Source: CAD feature listing. Evaluate the final solid. Frame: model axes, mm. Face numbers are marked on the shaded views. A direction names the side the tool comes from. Give positions to 0.01 mm unless a question says otherwise; leave off trailing zeros. Order: outer loops, then holes, each group sorted by start corner. A loop starts at its lowest first (then second) coordinate and runs counter-clockwise, first axis right, second up. Notation, with made-up numbers: M -30,-24.75 L -14,-24.75 A22 ccw -14,2.25 Z; hole C 0,61 d3. An arc over 180 degrees is marked long. Use CSV: the item, a comma, the result in double quotes. Start each with the question number.
Item 1: Section query B-B on y = 67. Return loops of the section in (x, z), and give its area (3 significant figures).
Item 2: Pull-direction query (X, two-part tool) for the marked faces 4, 5, 6 and 7; classes: +X half, -X half, draft (parallel to the pull), parting line (faces both ways), or undercut.
Item 3: Access query for the marked faces 1, 2 and 3. Directions: +Z, -Z, +X, -X, +Y, -Y. A direction counts if a zero-diameter tool reaches every point of the face in a straight line with its end or side. Return the directions, or none.
Item 4: Section query D-D on x = 133.5. Return loops of the section in (y, z).
Item 5: First-contact query: pin 1 (12 mm diameter, centred on x = 128.5, y = 21, fed in from -Z); pin 2 (18.5 mm diameter, centred on y = 20, z = 11.5, fed in from +X); pin 3 (15 mm diameter, centred on x = 144, z = 32.5, fed in from +Y); pin 4 (2 mm diameter, centred on x = 63.5, z = 54, fed in from +Y). Flat tips, straight axial feed; report the tip coordinate or a pass-through.
Item 6: Ray query, probe 1 along Z at (x, y) = (62.5, 22.5); probe 2 along Z at (x, y) = (96.5, 29.5); probe 3 along Y at (x, z) = (90, 66). Return the intervals inside material, ascending. Write a range as from..to.
Item 7: Section query C-C on x = 80.5. Return loops of the section in (y, z).
Item 8: Section query A-A on z = 41. Return loops of the section in (x, y), and give its area (4 significant figures).
from build123d import *

# Parameters (mm, degrees)
BASE_BLOCK_DEPTH       = 82
POCKET_1_SKETCH_W      = 82
POCKET_1_SKETCH_H      = 15
POCKET_CUT_1_DEPTH     = 82
POCKET_2_SKETCH_W      = 12
POCKET_2_SKETCH_H      = 82
POCKET_CUT_2_DEPTH     = 82
PAD_SKETCH_W           = 12
PAD_SKETCH_H           = 15
FULL_WIDTH_PAD_DEPTH   = 82
LUG_1_DEPTH            = 22
LUG_START              = -22
LUG_2_DEPTH            = 22
WEB_1_DEPTH            = 12
WEB_2_DEPTH            = 12
WEB_3_DEPTH            = 12
WEB_4_DEPTH            = 12
LUG_BORE_SKETCH_R      = 14
LUG_BORE_DEPTH         = 100
EAR_BOSS_DEPTH         = 15
EAR_HOLE_SKETCH_R      = 11
EAR_HOLE_DEPTH         = 15
SIDE_BOSS_DEPTH        = 10
BEARING_SEAT_CUT_DEPTH = 28


with BuildPart() as part:
    # Base Profile Sketch → Base Block (new body)
    with BuildSketch(Plane.XY):
        Polygon((0, 15), (0, 0), (140, 0), (140, 30), (128, 30), (128, 15), (18, 14), (18, 54), (0, 54), align=None)
    extrude(amount=BASE_BLOCK_DEPTH)

    # Pocket 1 Sketch → Pocket Cut 1 (cut)
    with BuildSketch(Plane.ZY.offset(-128)):
        with Locations((41, 22.5)):
            Rectangle(POCKET_1_SKETCH_W, POCKET_1_SKETCH_H)
    extrude(amount=-POCKET_CUT_1_DEPTH, mode=Mode.SUBTRACT)

    # Pocket 2 Sketch → Pocket Cut 2 (cut)
    with BuildSketch(Plane(origin=(0, 15, 0), x_dir=(1, 0, 0), z_dir=(0, 1, 0))):
        with Locations((134, -41)):
            Rectangle(POCKET_2_SKETCH_W, POCKET_2_SKETCH_H)
    extrude(amount=-POCKET_CUT_2_DEPTH, mode=Mode.SUBTRACT)

    # Pad Sketch → Full Width Pad (add)
    with BuildSketch(Plane.XY.offset(82)):
        with Locations((134, 7.5)):
            Rectangle(PAD_SKETCH_W, PAD_SKETCH_H)
    extrude(amount=-FULL_WIDTH_PAD_DEPTH)

    # Lug 1 Sketch → Lug 1 (add)
    with BuildSketch(Plane.XY.offset(82)):
        with BuildLine():
            ThreePointArc((115, 65), (90, 90), (65, 65))
            Line((65, 65), (65, 14.427272727))
            Line((65, 14.427272727), (90, 14.654545455))
            Line((90, 14.654545455), (115, 14.881818182))
            Line((115, 14.881818182), (115, 65))
        make_face()
    extrude(amount=-LUG_1_DEPTH)

    # Lug 2 Sketch → Lug 2 (add)
    with BuildSketch(Plane(origin=(0, 0, 0), x_dir=(-1, 0, 0), z_dir=(0, 0, -1)).offset(LUG_START)):
        with BuildLine():
            Line((-115, 65), (-115, 14.881818182))
            Line((-115, 14.881818182), (-65, 14.427272727))
            Line((-65, 14.427272727), (-65, 65))
            ThreePointArc((-65, 65), (-90, 90), (-115, 65))
        make_face()
    extrude(amount=LUG_2_DEPTH)

    # Web 1 Sketch → Web 1 (add)
    with BuildSketch(Plane(origin=(0, 0, 0), x_dir=(-1, 0, 0), z_dir=(0, 0, -1))):
        Polygon((-18, 14), (-18, 29), (-65, 29), (-65, 14.427272727), align=None)
    extrude(amount=-WEB_1_DEPTH)

    # Web 2 Sketch → Web 2 (add)
    with BuildSketch(Plane(origin=(0, 0, 0), x_dir=(-1, 0, 0), z_dir=(0, 0, -1))):
        Polygon((-140, 15), (-140, 30), (-115, 30), (-115, 14.881818182), align=None)
    extrude(amount=-WEB_2_DEPTH)

    # Web 3 Sketch → Web 3 (add)
    with BuildSketch(Plane.XY.offset(82)):
        Polygon((115, 30), (115, 14.881818182), (140, 15), (140, 30), align=None)
    extrude(amount=-WEB_3_DEPTH)

    # Web 4 Sketch → Web 4 (add)
    with BuildSketch(Plane.XY.offset(82)):
        Polygon((18, 14), (18, 29), (65, 29), (65, 14.427272727), align=None)
    extrude(amount=-WEB_4_DEPTH)

    # Lug Bore Sketch → Lug Bore (cut)
    with BuildSketch(Plane.XY.offset(82)):
        with Locations((90, 65)):
            Circle(LUG_BORE_SKETCH_R)
    extrude(amount=-LUG_BORE_DEPTH, mode=Mode.SUBTRACT)

    # Ear Boss Sketch → Ear Boss (add)
    with BuildSketch(Plane(origin=(0, 15, 0), x_dir=(1, 0, 0), z_dir=(0, 1, 0))):
        with BuildLine():
            Line((140, -23), (140, -59))
            ThreePointArc((140, -59), (158, -41), (140, -23))
        make_face()
    extrude(amount=-EAR_BOSS_DEPTH)

    # Ear Hole Sketch → Ear Hole (cut)
    with BuildSketch(Plane(origin=(0, 15, 0), x_dir=(1, 0, 0), z_dir=(0, 1, 0))):
        with Locations(Location((140, -41, 0), (0, 0, 270))):
            Circle(EAR_HOLE_SKETCH_R)
    extrude(amount=-EAR_HOLE_DEPTH, mode=Mode.SUBTRACT)

    # Side Boss Sketch → Side Boss (add)
    with BuildSketch(Plane(origin=(18, 0, 0), x_dir=(0, 0, -1), z_dir=(1, 0, 0))):
        with BuildLine():
            Line((-63, 54), (-19, 54))
            ThreePointArc((-19, 54), (-41, 32), (-63, 54))
        make_face()
    extrude(amount=SIDE_BOSS_DEPTH)

    # Bearing Seat Sketch → Bearing Seat Cut (cut)
    with BuildSketch(Plane.ZY):
        with BuildLine():
            Line((27, 54), (55, 54))
            ThreePointArc((55, 54), (41, 40), (27, 54))
        make_face()
    extrude(amount=-BEARING_SEAT_CUT_DEPTH, mode=Mode.SUBTRACT)


solid = part.part
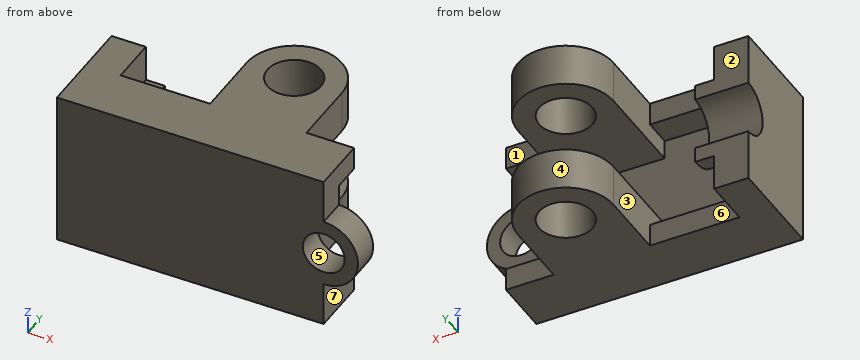
Verdict:
1,outline,"M 65.08,0 L 76.14,0 L 76.14,22 L 65.08,22 Z; M 65.08,60 L 76.14,60 L 76.14,82 L 65.08,82 Z; M 103.86,0 L 114.92,0 L 114.92,22 L 103.86,22 Z; M 103.86,60 L 114.92,60 L 114.92,82 L 103.86,82 Z"
1,area,"974 mm2"
2,face 4,"parting line"
2,face 5,"undercut"
2,face 6,"undercut"
2,face 7,"+X half"
3,face 1,"+Z, -Z, +X, +Y"
3,face 2,"+Z, -Z, -X, +Y"
3,face 3,"+Y"
4,outline,"M 0,0 L 30,0 L 30,12 L 15,12 L 15,32.13 L 0,32.13 Z; M 0,49.87 L 15,49.87 L 15,70 L 30,70 L 30,82 L 0,82 Z"
5,pin 1,"z = 0"
5,pin 2,"x = 140"
5,pin 3,"y = 15"
5,pin 4,"y = 14.42"
6,probe 1,"0..12, 70..82"
6,probe 2,"0..22, 60..82"
6,probe 3,"0..51, 79..90"
7,outline,"M 0,0 L 54.72,0 L 54.72,22 L 14.57,22 L 14.57,60 L 54.72,60 L 54.72,82 L 0,82 Z; M 75.28,0 L 88.12,0 L 88.12,22 L 75.28,22 Z; M 75.28,60 L 88.12,60 L 88.12,82 L 75.28,82 Z"
8,outline,"M 0,0 L 129,0 L 129,15 L 128,15 L 18,14 L 18,32 L 28,32 L 28,40 L 0,40 Z; M 151,0 L 158,0 L 158,15 L 151,15 Z"
8,area,"2,515 mm2"
